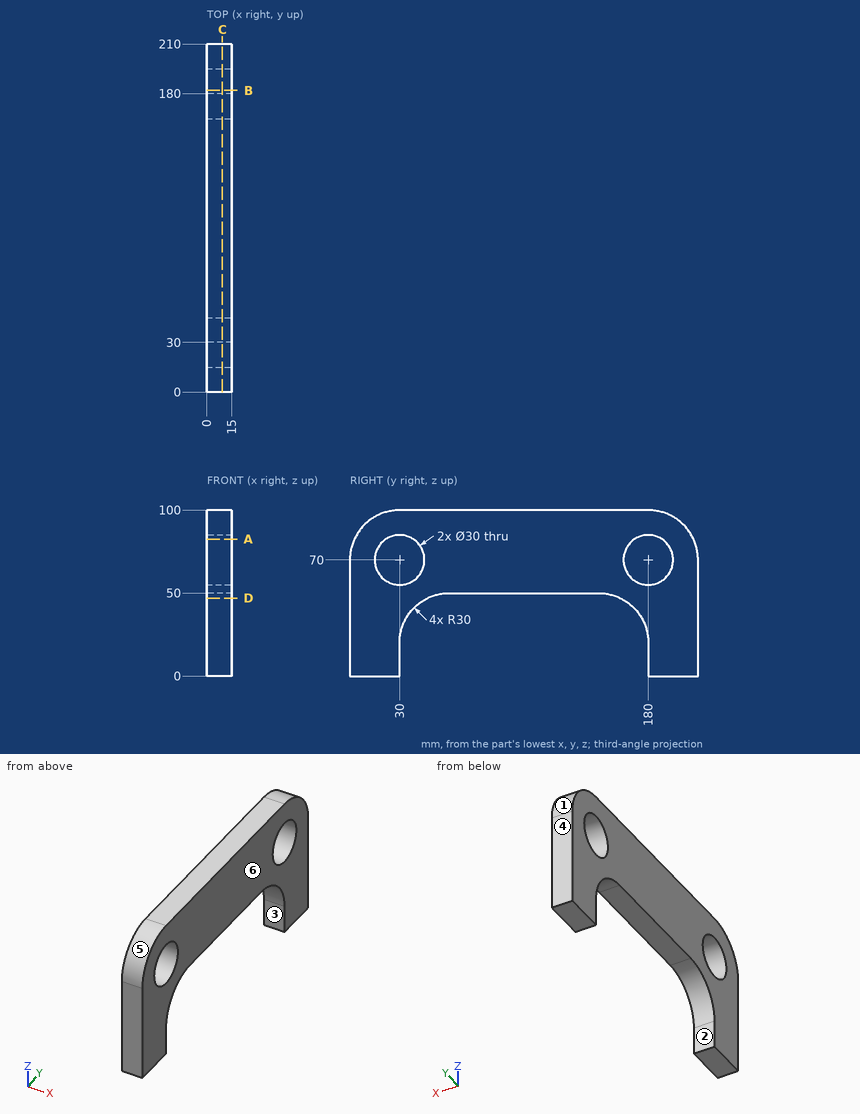
Part print with two shaded views. Sizes in mm from the minimum x, y, z corner. A direction names the side the tool comes from. Give positions to 0.01 mm unless a question says otherwise; leave off trailing zeros. Order: outer loops, then holes, each group sorted by start corner. A loop starts at its lowest first (then second) coordinate and runs counter-clockwise, first axis right, second up. Notation, with made-up numbers: M 30,68.5 L 85,68.5 A23 cw 85,76.5 Z; hole C 25.25,10.25 d4. An arc over 180 degrees is marked long. Put each result on its own line as item: value.
Item 1: Cut at D-D on z = 47. Write the cut outline in (x, y).
Results are:
outline: M 0,0 L 15,0 L 15,46.92 L 0,46.92 Z; M 0,163.08 L 15,163.08 L 15,210 L 0,210 Z
Item 2: Pull direction Y, two halves, no side cores. Call the marked faces 3, 4, 5 and 6: +Y half, -Y half, draft (parallel to the pull), parting line (faces both ways), or undercut.
Results are:
face 3: undercut
face 4: +Y half
face 5: -Y half
face 6: draft
Item 3: Cut at C-C on x = 9.25. Write the cut outline in (y, z).
Results are:
outline: M 0,0 L 30,0 L 30,20 A30 cw 60,50 L 150,50 A30 cw 180,20 L 180,0 L 210,0 L 210,70 A30 ccw 180,100 L 30,100 A30 ccw 0,70 Z; hole C 30,70 d30; hole C 180,70 d30
Item 4: Drop flat-ended pins along their axis: pin 1 Ø6 at (x, y) = (6.5, 111.5) entering from -Z; pin 2 Ø4 at (y, z) = (187.5, 87) entering from -X; pin 3 Ø18 at (y, z) = (180, 70) entering from -X. Give the stop position or say it passes through.
Results are:
pin 1: z = 50
pin 2: x = 0
pin 3: through
Item 5: Cut at B-B on y = 182. Write the cut outline in (x, z).
Results are:
outline: M 0,0 L 15,0 L 15,55.13 L 0,55.13 Z; M 0,84.87 L 15,84.87 L 15,99.93 L 0,99.93 Z
Item 6: Which spindle directions (+Z, -Z, +X, -X, +Y, -Y) get a long thin tool onto all of the face, cutting with end or side? Do the marked faces 1 and 2. Say none if no direction does.
Results are:
face 1: +Z, +X, -X, +Y
face 2: -Z, +X, -X
Item 7: Wall check: probe 1 along Y at (x, z) = (12, 70); probe 2 along Y at (x, z) = (9, 7); probe 3 along Y at (x, z) = (6, 73.5). Give the ranges that are in metal, low to high.
Results are:
probe 1: 0 to 15, 45 to 165, 195 to 210
probe 2: 0 to 30, 180 to 210
probe 3: 0.2 to 15.41, 44.59 to 165.41, 194.59 to 209.8
Item 8: Cut at A-A on z = 82.5. Write the cut outline in (x, y), then the cut area to 3 significant figures.
Results are:
outline: M 0,2.73 L 15,2.73 L 15,21.71 L 0,21.71 Z; M 0,38.29 L 15,38.29 L 15,171.71 L 0,171.71 Z; M 0,188.29 L 15,188.29 L 15,207.27 L 0,207.27 Z
area: 2,570 mm2
